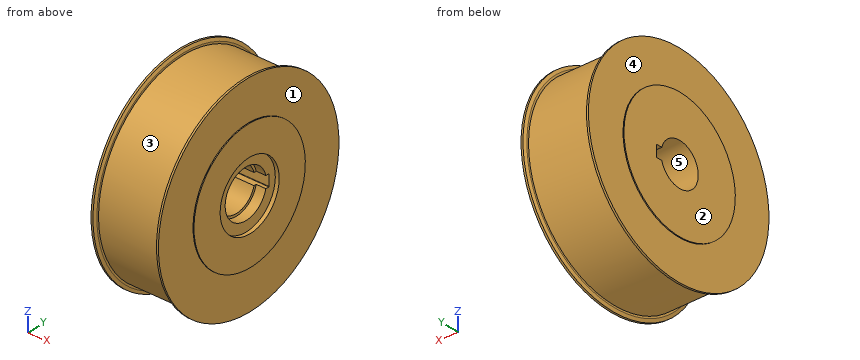
```python
from build123d import *

# Parameters (mm, degrees)
SKETCH2_R          = 17.5
CUT_EXTRUDE1_DEPTH = 2
CUT_EXTRUDE2_DEPTH = 83.948779376
SKETCH4_R          = 12.25
CUT_EXTRUDE3_DEPTH = 5
FILLET1_R          = 0.2


with BuildPart() as part:
    # Sketch1 → Revolve1 (revolve)
    with BuildSketch(Plane.XY, mode=Mode.PRIVATE) as revolve1_sk:
        Polygon((-18, 0), (-18, 33), (-17.5, 33), (-17.5, 53.5), (-16.5, 53.5), (-15.9, 51.9), (-15.9, 50.9), (15.9, 50.9), (15.9, 51.9), (16.5, 53.5), (17.5, 53.5), (17.5, 33), (18, 33), (18, 0), align=None)
    revolve(revolve1_sk.sketch.rotate(Axis((-18, 0, 0), (1, 0, 0)), 90), axis=Axis((-18, 0, 0), (1, 0, 0)))

    # Sketch2 → Cut-Extrude1 (cut)
    with BuildSketch(Plane(origin=(18, 0, 0), x_dir=(0, 0, -1), z_dir=(1, 0, 0))):
        Circle(SKETCH2_R)
    extrude(amount=-CUT_EXTRUDE1_DEPTH, mode=Mode.SUBTRACT)

    # Sketch3 → Cut-Extrude2 (cut, through all)
    with BuildSketch(Plane(origin=(16, 0, 0), x_dir=(0, 0, -1), z_dir=(1, 0, 0))):
        with BuildLine():
            Line((3, 10.583005244), (3, 13.8))
            Line((3, 13.8), (-3, 13.8))
            Line((-3, 13.8), (-3, 10.583005244))
            ThreePointArc((-3, 10.583005244), (0, -11), (3, 10.583005244))
        make_face()
    extrude(amount=-CUT_EXTRUDE2_DEPTH, mode=Mode.SUBTRACT)

    # Sketch4 → Cut-Extrude3 (cut)
    with BuildSketch(Plane(origin=(16, 0, 0), x_dir=(0, 0, -1), z_dir=(1, 0, 0))):
        Circle(SKETCH4_R)
    extrude(amount=-CUT_EXTRUDE3_DEPTH, mode=Mode.SUBTRACT)

    # Fillet1
    fillet1_edges = [part.edges().sort_by_distance(p)[0] for p in [
        (-1, 13.8, 3),
        (-1, 13.8, -3),
    ]]
    fillet(fillet1_edges, radius=FILLET1_R)


solid = part.part
```
Here's how the part is built. I have some questions about the finished solid (model axes, mm). Face numbers are marked on the shaded views. A direction names the side the tool comes from. Round coordinates to 2 decimals unless told otherwise and drop trailing zeros. Write each loop counter-clockwise with the first axis right and the second up, starting at its lowest first coordinate (ties: lowest second). Pieces come first, ordered by that corner, then holes. Notation, with made-up numbers: M 82,59 L 90,59 A18 ccw 90,88 Z; hole C -14,10 d9. An arc over 180 degrees is marked long. Answer as CSV lines item,"result". Start each with the question number.
1. I need wall thicknesses on probe 1 along Y at (x, z) = (3, 0); probe 2 along Y at (x, z) = (12.8, 0); probe 3 along X at (y, z) = (-24.5, -45). Which ranges of each line are inside material? Lowest first, please.
2. Suppose I cut it at B-B on x = 13. Write out the boundary of the cut face in (y, z), then the cut area to 3 significant figures.
3. On a 3-axis mill with a long thin cutter (end or side, diameter ignored), from which of +Z, -Z, +X, -X, +Y, -Y can I reach the whole of each face in a straight line? I mean the marked faces 1 and 2. Say none if no direction works.
4. Suppose I cut it at C-C on x = -8.5. Write out the boundary of the cut face in (y, z), then the cut area to 3 significant figures.
5. Thinking about a two-plate mould opening in X: for the marked faces 3, 4 and 5, which applies, released by +X, released by -X, zero draft, split by the parting line, or undercut?
6. I'm going to push flat-ended pins straight in: pin 1 Ø10 at (x, y) = (14, -20) entering from -Z; pin 2 Ø17.5 at (y, z) = (-5.5, -3) entering from +X; pin 3 Ø1.5 at (x, y) = (5.5, 11.5) entering from +Z. Where does each tip first touch, or does it pass through?
Check result:
1,probe 1,"y = -50.9 to -11, 13.8 to 50.9"
1,probe 2,"y = -50.9 to -12.25, 13.8 to 50.9"
1,probe 3,"x = -17.5 to -15.9, 15.9 to 17.5"
2,outline,"C 0,0 d101.8; hole M 11.88,-3 L 13.6,-3 A0.2 ccw 13.8,-2.8 L 13.8,2.8 A0.2 ccw 13.6,3 L 11.88,3 A12.25 ccw long Z"
2,area,"7,660 mm2"
3,face 1,"+X"
3,face 2,"+Z, -Z, -X, +Y, -Y"
4,outline,"C 0,0 d101.8; hole M 10.58,-3 L 13.6,-3 A0.2 ccw 13.8,-2.8 L 13.8,2.8 A0.2 ccw 13.6,3 L 10.58,3 A11 ccw long Z"
4,area,"7,740 mm2"
5,face 3,"undercut"
5,face 4,"released by -X"
5,face 5,"zero draft"
6,pin 1,"stops at z = -51.15"
6,pin 2,"stops at x = 16"
6,pin 3,"stops at z = 49.75"
